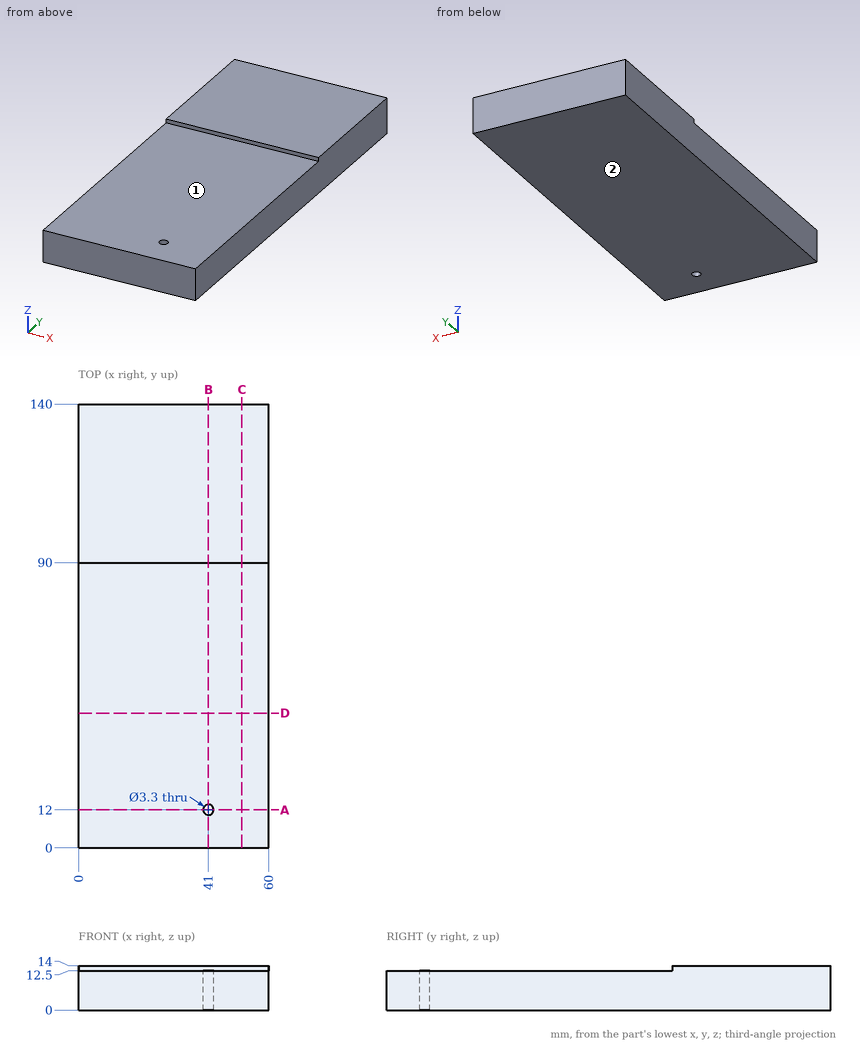
The figure shows three views and two pictorial views of one solid part (mm, origin at its lowest corner). Answer the questions. A direction names the side the tool comes from. Round coordinates to 2 decimals unless told otherwise and drop trailing zeros. Loops run counter-clockwise (first coordinate to the right, second up) from the corner with the lowest first, then second, coordinate; pieces in that order, holes last. Notation, with made-up numbers: (-4.5, 51.5) -> (9.5, 51.5) arc R15 cw to (9.5, 63.5) -> close; hole circle Ø4 at (-25.75, 55). An arc over 180 degrees is marked (long way). Use one line per item in the form item = value.
(1) Straight lines are drawn through the part: line 1 (Y direction, x = 41, z = 5.25); line 2 (Z direction, x = 22, y = 75); line 3 (Y direction, x = 47.5, z = 13.25). For each, find the intervals that lie inside material, in ascending order.
Answer list:
line_1 = 0 to 10.35, 13.65 to 140
line_2 = 0 to 12.5
line_3 = 90 to 140
(2) A tool of negligible diameter and unlimited length cuts with its end or side. For the marked faces 1 and 2, from which of +Z, -Z, +X, -X, +Y, -Y can it reach the whole face along a straight path? Write none if from no direction.
Answer list:
face_1 = +Z, +X, -X, -Y
face_2 = -Z, +X, -X, +Y, -Y
(3) Find section B-B on x = 41. Give the vertices of the cut face in (y, z), then the cut area to 3 significant figures.
Answer list:
outline = (0, 0) -> (10.35, 0) -> (10.35, 12.5) -> (0, 12.5) -> close; (13.65, 0) -> (140, 0) -> (140, 14) -> (90, 14) -> (90, 12.5) -> (13.65, 12.5) -> close
area = 1,780 mm2
(4) A flat-ended cylindrical pin translates along its axis: P1, Ø1.5, axis at x = 26, y = 72.5, coming from the +Z side. Find the tip coordinate at first contact, or state that the pin passes through.
Answer list:
P1 = 12.5
(5) Find section A-A on y = 12. Give the vertices of the cut face in (x, z).
Answer list:
outline = (0, 0) -> (39.35, 0) -> (39.35, 12.5) -> (0, 12.5) -> close; (42.65, 0) -> (60, 0) -> (60, 12.5) -> (42.65, 12.5) -> close
(6) Find section C-C on x = 51.5. Give the vertices of the cut face in (y, z), then the cut area to 4 significant figures.
Answer list:
outline = (0, 0) -> (140, 0) -> (140, 14) -> (90, 14) -> (90, 12.5) -> (0, 12.5) -> close
area = 1,825 mm2
(7) Find section D-D on y = 42.5. Give the vertices of the cut face in (x, z).
Answer list:
outline = (0, 0) -> (60, 0) -> (60, 12.5) -> (0, 12.5) -> close
